```python
from build123d import *

# Parameters (mm, degrees)
SKETCH_1_W                  = 165
SKETCH_1_H                  = 600
EXTRUDE_1_DEPTH             = 10
SKETCH_5_R                  = 15
CUT_EXTRUDE_1_DEPTH         = 322.442063209
HOLE_WIZARD_M4_1_D          = 3.3
HOLE_WIZARD_M3_1_D          = 2.5
HOLE_WIZARD_M4_3_D          = 3.3
SKETCH_18_R                 = 7
CUT_EXTRUDE_2_DEPTH         = 322.442063209
HOLE_WIZARD_M4_4_D          = 3.3
HOLE_WIZARD_M4_4_DEPTH      = 10
HOLE_WIZARD_M4_4_TIP        = 0.991420021
HOLE_WIZARD_M4_5_D          = 3.3
HOLE_WIZARD_M4_5_DEPTH      = 10.1
HOLE_WIZARD_M4_5_TIP        = 0.991420021
HOLE_WIZARD_6_D             = 4.5
HOLE_WIZARD_6_CBORE_D       = 8
HOLE_WIZARD_6_CBORE_DEPTH   = 4.6
SKETCH_27_W                 = 71.16849895
SKETCH_27_H                 = 73
CUT_EXTRUDE_3_DEPTH         = 322.442063209
HOLE_WIZARD_5_D             = 4.5
HOLE_WIZARD_5_CBORE_D       = 8
HOLE_WIZARD_5_CBORE_DEPTH   = 4.6
HOLE_WIZARD_6_2_D           = 6.6
HOLE_WIZARD_6_2_CBORE_D     = 11
HOLE_WIZARD_6_2_CBORE_DEPTH = 6.8


with BuildPart() as part:
    # 草图1 → 凸台-拉伸1 (new body)
    with BuildSketch(Plane.XY):
        with Locations((-32.5, 0)):
            Rectangle(SKETCH_1_W, SKETCH_1_H)
    extrude(amount=EXTRUDE_1_DEPTH)

    # 草图5 → 切除-拉伸1 (cut, through all)
    with BuildSketch(Plane.XY.offset(10)):
        with Locations((-5, 100)):
            Circle(SKETCH_5_R)
    extrude(amount=-CUT_EXTRUDE_1_DEPTH, mode=Mode.SUBTRACT)

    # M4 螺纹孔1 (through all)
    with Locations(Plane.XY.offset(10)):
        with Locations((-66, -120), (-1, -98), (-1, -120), (-66, -98)):
            Hole(HOLE_WIZARD_M4_1_D / 2)

    # M3 螺纹孔1 (through all)
    with Locations(Plane.XY.offset(10)):
        with Locations((-10, 41.3), (10, 41.3)):
            Hole(HOLE_WIZARD_M3_1_D / 2)

    # M4 螺纹孔3 (through all)
    with Locations(Plane(origin=(0, 0, 0), x_dir=(-1, 0, 0), z_dir=(0, 0, -1))):
        with Locations((107.75, 193.999999998), (107.75, -194.000000002)):
            Hole(HOLE_WIZARD_M4_3_D / 2)

    # 草图18 → 切除-拉伸2 (cut, through all)
    with BuildSketch(Plane(origin=(0, 0, 0), x_dir=(-1, 0, 0), z_dir=(0, 0, -1))):
        with Locations((-24, 187.5)):
            Circle(SKETCH_18_R)
        with Locations((-24, -187.5)):
            Circle(SKETCH_18_R)
    extrude(amount=-CUT_EXTRUDE_2_DEPTH, mode=Mode.SUBTRACT)

    # M4 螺纹孔4
    with Locations(Plane(origin=(0, -300, 0), x_dir=(-1, 0, 0), z_dir=(0, -1, 0))):
        with Locations((-10, -4), (85, -4)):
            Hole(HOLE_WIZARD_M4_4_D / 2, depth=HOLE_WIZARD_M4_4_DEPTH)
            with Locations((0, 0, -(HOLE_WIZARD_M4_4_DEPTH + HOLE_WIZARD_M4_4_TIP / 2))):  # 118° drill point
                Cone(0, HOLE_WIZARD_M4_4_D / 2, HOLE_WIZARD_M4_4_TIP, mode=Mode.SUBTRACT)

    # M4 螺纹孔5
    with Locations(Plane(origin=(0, 300, 0), x_dir=(1, 0, 0), z_dir=(0, 1, 0))):
        with Locations((-85, -4), (10, -4)):
            Hole(HOLE_WIZARD_M4_5_D / 2, depth=HOLE_WIZARD_M4_5_DEPTH)
            with Locations((0, 0, -(HOLE_WIZARD_M4_5_DEPTH + HOLE_WIZARD_M4_5_TIP / 2))):  # 118° drill point
                Cone(0, HOLE_WIZARD_M4_5_D / 2, HOLE_WIZARD_M4_5_TIP, mode=Mode.SUBTRACT)

    # Hole Wizard 6 (through all)
    with Locations(Plane.XY.offset(10)):
        with Locations((43, 262), (43, 82), (43, -82), (43, -262)):
            CounterBoreHole(HOLE_WIZARD_6_D / 2, HOLE_WIZARD_6_CBORE_D / 2, HOLE_WIZARD_6_CBORE_DEPTH)

    # 草图27 → 切除-拉伸3 (cut, through all)
    with BuildSketch(Plane(origin=(0, 0, 0), x_dir=(-1, 0, 0), z_dir=(0, 0, -1))):
        with Locations((88.584249475, 109.5)):
            Rectangle(SKETCH_27_W, SKETCH_27_H)
    extrude(amount=-CUT_EXTRUDE_3_DEPTH, mode=Mode.SUBTRACT)

    # 打孔尺寸根据内六角圆柱头螺钉的类型5 (through all)
    with Locations(Plane.XY.offset(10)):
        with Locations((-80, 240), (-80, 210)):
            CounterBoreHole(HOLE_WIZARD_5_D / 2, HOLE_WIZARD_5_CBORE_D / 2, HOLE_WIZARD_5_CBORE_DEPTH)

    # Hole Wizard 6 2 (through all)
    with Locations(Plane(origin=(0, 0, 0), x_dir=(-1, 0, 0), z_dir=(0, 0, -1))):
        with Locations((30.000000001, 285), (-35, 285), (30.000000001, 2e-09), (30.000000001, -284.999999998), (-35, -284.999999998)):
            CounterBoreHole(HOLE_WIZARD_6_2_D / 2, HOLE_WIZARD_6_2_CBORE_D / 2, HOLE_WIZARD_6_2_CBORE_DEPTH)


solid = part.part
```
Source: CAD feature listing. Evaluate the final solid. Frame: model axes, mm. A direction names the side the tool comes from. Give positions to 0.01 mm unless a question says otherwise; leave off trailing zeros. Order: outer loops, then holes, each group sorted by start corner. A loop starts at its lowest first (then second) coordinate and runs counter-clockwise, first axis right, second up. Notation, with made-up numbers: (31.5, 2) -> (67.5, 2) arc R8 ccw to (67.5, 6) -> close; hole circle Ø2 at (65.25, -25). An arc over 180 degrees is marked (long way). Use a Markdown table: item, result.
Q1. Section B-B (x = 24). Return the cut outline in (y, z).
A:
| item | result |
|---|---|
| outline | (-300, 0) -> (-194.5, 0) -> (-194.5, 10) -> (-300, 10) -> close; (-180.5, 0) -> (180.5, 0) -> (180.5, 10) -> (-180.5, 10) -> close; (194.5, 0) -> (300, 0) -> (300, 10) -> (194.5, 10) -> close |
Q2. Access query for faces 4 (the face through (-24.505, 0.242, 3.352)), 5 (the face through (-84, 146, 5)), 6 (the face through (-115, 222, 5)). Directions: +Z, -Z, +X, -X, +Y, -Y. A direction counts if a zero-diameter tool reaches every point of the face in a straight line with its end or side. Return the directions, or none.
A:
| item | result |
|---|---|
| face 4 | -Z |
| face 5 | +Z, -Z, -X |
| face 6 | +Z, -Z, -X, +Y, -Y |
Q3. Section A-A (y = 100). Return the cut outline in (x, z).
A:
| item | result |
|---|---|
| outline | (-53, 0) -> (-20, 0) -> (-20, 10) -> (-53, 10) -> close; (10, 0) -> (50, 0) -> (50, 10) -> (10, 10) -> close |
Q4. Pull-direction query (Y, two-part tool) for faces 1 (the face through (-34, 300, 5)), 2 (the face through (-28.81, 279.63, 3.35)), 3 (the face through (50, -4, 5)); classes: +Y half, -Y half, draft (parallel to the pull), parting line (faces both ways), or undercut.
A:
| item | result |
|---|---|
| face 1 | +Y half |
| face 2 | undercut |
| face 3 | draft |
Q5. Material intervals for line 1 (Y direction, x = -30, z = 2.5); line 2 (Y direction, x = 43, z = 8.65); line 3 (Y direction, x = -80, z = 3.5), sorted ascending. Write a range as [from, to].
A:
| item | result |
|---|---|
| line 1 | [-300, -290.5], [-279.5, -5.5], [5.5, 279.5], [290.5, 300] |
| line 2 | [-300, -266], [-258, -86], [-78, 78], [86, 258], [266, 300] |
| line 3 | [-300, 73], [146, 207.75], [212.25, 237.75], [242.25, 300] |
Q6. First-contact query: P1, Ø7, axis at x = -80, y = 240, coming from the +Z side; P2, Ø2.5, axis at x = -85, z = 4, coming from the -Y side; P3, Ø2.5, axis at x = 10, z = 4, coming from the +Y side. Flat tips, straight axial feed; report the tip coordinate or a pass-through.
A:
| item | result |
|---|---|
| P1 | z = 5.4 |
| P2 | y = -289.76 |
| P3 | y = 289.66 |
